Could you check a few things on this model? Use its own coordinates, in mm. A direction names the side the tool comes from. Give positions to 0.01 mm unless a question says otherwise; leave off trailing zeros. Order: outer loops, then holes, each group sorted by start corner. A loop starts at its lowest first (then second) coordinate and runs counter-clockwise, first axis right, second up. Notation, with made-up numbers: (4, 22.25) -> (50, 22.25) arc R15 cw to (50, 27.25) -> close; hole circle Ø6 at (68, 30.5). An arc over 180 degrees is marked (long way). One line per item, written item: value.
```python
from build123d import *

# Parameters (mm, degrees)
EXTRUDE_1_DEPTH     = 205
SHELL_1_T           = -2
SKETCH_4_W          = 1600
SKETCH_4_H          = 205
SKETCH_4_W_2        = 1540
SKETCH_4_H_2        = 145
EXTRUDE_2_DEPTH     = 2
SKETCH_5_R          = 4.5
CUT_EXTRUDE_1_DEPTH = 2
SKETCH_7_R          = 4.5
CUT_EXTRUDE_2_DEPTH = 78
SKETCH_8_R          = 4.5
CUT_EXTRUDE_3_DEPTH = 16
SKETCH_9_R          = 4.5
CUT_EXTRUDE_4_DEPTH = 110


with BuildPart() as part:
    # 草图2 → 凸台-拉伸1 (new body)
    with BuildSketch(Plane(origin=(0, 0, 0), x_dir=(-1, 0, 0), z_dir=(0, 0, -1))):
        Polygon((-1600, -30), (-1500.029639528, -100), (-787, -100), (-707.152509296, -167), (0, -167), (0, 0), (-1600, 0), align=None)
    extrude(amount=EXTRUDE_1_DEPTH)

    # 抽壳1
    shell_1_openings = [part.faces().sort_by_distance(p)[0] for p in [
        (800, 0, -102.5),
    ]]
    offset(amount=SHELL_1_T, openings=shell_1_openings, kind=Kind.INTERSECTION)

    # 草图4 → 凸台-拉伸2 (add)
    with BuildSketch(Plane(origin=(0, 0, 0), x_dir=(1, 0, 0), z_dir=(0, 1, 0))):
        with Locations((800, 102.5)):
            Rectangle(SKETCH_4_W, SKETCH_4_H)
        with Locations((800, 102.5)):
            Rectangle(SKETCH_4_W_2, SKETCH_4_H_2, mode=Mode.SUBTRACT)
    extrude(amount=-EXTRUDE_2_DEPTH)

    # 草图5 → 切除-拉伸1 (cut)
    with BuildSketch(Plane(origin=(0, 0, -205), x_dir=(-1, 0, 0), z_dir=(0, 0, -1))):
        with Locations((-1570, -14)):
            Circle(SKETCH_5_R)
        with Locations((-30, -14)):
            Circle(SKETCH_5_R)
        with Locations((-800, -14)):
            Circle(SKETCH_5_R)
    extrude(amount=-CUT_EXTRUDE_1_DEPTH, mode=Mode.SUBTRACT)

    # 草图7 → 切除-拉伸2 (cut)
    with BuildSketch(Plane.ZY):
        with Locations((-175, -151)):
            Circle(SKETCH_7_R)
        with Locations((-30, -151)):
            Circle(SKETCH_7_R)
    extrude(amount=-CUT_EXTRUDE_2_DEPTH, mode=Mode.SUBTRACT)

    # 草图8 → 切除-拉伸3 (cut)
    with BuildSketch(Plane(origin=(0, 0, 0), x_dir=(1, 0, 0), z_dir=(0, 1, 0))):
        with Locations(Location((1584, 175, 0), (0, 0, 180))):
            Circle(SKETCH_8_R)
        with Locations(Location((1584, 30, 0), (0, 0, 180))):
            Circle(SKETCH_8_R)
    extrude(amount=-CUT_EXTRUDE_3_DEPTH, mode=Mode.SUBTRACT)

    # 草图9 → 切除-拉伸4 (cut)
    with BuildSketch(Plane.XY):
        with Locations((817, -84)):
            Circle(SKETCH_9_R)
        with Locations((1470.029639528, -84)):
            Circle(SKETCH_9_R)
    extrude(amount=-CUT_EXTRUDE_4_DEPTH, mode=Mode.SUBTRACT)


solid = part.part
```
1) Suppose I cut it at D-D, the plane x = 834.5. Write out the boundary of the cut face in (y, z).
Answer below:
outline: (-100, -205) -> (0, -205) -> (0, -175) -> (-2, -175) -> (-2, -203) -> (-98, -203) -> (-98, -2) -> (-2, -2) -> (-2, -30) -> (0, -30) -> (0, 0) -> (-100, 0) -> close
2) If I drill on line 1 along Y through (x, z) = (1.2, -30); line 2 along Y through (x, z) = (235.5, -194.5); line 3 along Z through (x, y) = (604, -23), over which ranges is the centre line in solid material (lowest first)?
Answer below:
line 1: y = -167 to -155.5, -146.5 to 0
line 2: y = -167 to -165, -2 to 0
line 3: z = -205 to -203, -2 to 0
3) Suppose I cut it at C-C, the plane y = -45. Write out the boundary of the cut face in (x, z).
Answer below:
outline: (0, -205) -> (1578.58, -205) -> (1578.58, 0) -> (0, 0) -> close; hole (2, -203) -> (1575.09, -203) -> (1575.09, -2) -> (2, -2) -> close
4) Suppose I cut it at A-A, the plane x = 138.5. Write out the boundary of the cut face in (y, z).
Answer below:
outline: (-167, -205) -> (0, -205) -> (0, -175) -> (-2, -175) -> (-2, -203) -> (-165, -203) -> (-165, -2) -> (-2, -2) -> (-2, -30) -> (0, -30) -> (0, 0) -> (-167, 0) -> close
5) We'd pull the mould along X, two halves only. Please class faces 1 (the flat face through (1600, -15, -101)), 2 (the flat face through (737, 0, -178)), 3 (the flat face through (2, -85, -101)): +X half, -X half, draft (parallel to the pull), parting line (faces both ways), or undercut.
Answer below:
face 1: +X half
face 2: draft
face 3: undercut
6) For P1, Ø7, axis at x = 1470.03, y = -84, coming from the +Z side; P2, Ø8, axis at x = 631.5, z = -83.5, coming from the +Y side; P3, Ø11.5, axis at y = -151, z = -30, coming from the +X side, each with a flat end and sliding along its axis, tell me the tip position at first contact or that it passes through.
Answer below:
P1: stops at z = -203
P2: stops at y = -165
P3: stops at x = 733.07
7) Suppose I cut it at B-B, the plane z = -80.5. Write out the boundary of the cut face in (x, y), then the cut area to 3 significant figures.
Answer below:
outline: (0, -167) -> (707.15, -167) -> (787, -100) -> (1500.03, -100) -> (1600, -30) -> (1600, 0) -> (1570, 0) -> (1570, -2) -> (1598, -2) -> (1598, -28.96) -> (1499.4, -98) -> (786.27, -98) -> (706.42, -165) -> (2, -165) -> (2, -2) -> (30, -2) -> (30, 0) -> (0, 0) -> close
area: 3,790 mm2
8) For faces 4 (the flat face through (359, -167, -101)), 5 (the flat face through (1149, -100, -101)), 6 (the flat face through (737, -2, -29)), which set-ups out of +Z, -Z, +X, -X, +Y, -Y let a thin tool reach every point of the face, with its end or its side?
Answer below:
face 4: +Z, -Z, +X, -X, -Y
face 5: +Z, -Z, +X, -Y
face 6: none
